```python
from build123d import *

# Parameters (mm, degrees)
CHAMFER1_SIZE  = 0.5
CHAMFER2_SIZE  = 1
CHAMFER2_SIZE2 = 0.3


with BuildPart() as part:
    # Sketch2 → Revolve1 (revolve)
    with BuildSketch(Plane.XY, mode=Mode.PRIVATE) as revolve1_sk:
        Polygon((4.5, 0), (4.5, 6), (4.9, 6), (4.9, 3), (6.25, 3), (6.25, 0), align=None)
    revolve(revolve1_sk.sketch.rotate(Axis((0, 0, 0), (0, 1, 0)), 90), axis=Axis((0, 0, 0), (0, 1, 0)))

    # Sketch3 → Cut-Revolve1 (revolve, cut)
    with BuildSketch(Plane.XY, mode=Mode.PRIVATE) as cut_revolve1_sk:
        Polygon((4.5, 3), (4.5, 0), (4.8, 0), align=None)
    revolve(cut_revolve1_sk.sketch.rotate(Axis((0, 0, 0), (0, 1, 0)), 90), axis=Axis((0, 0, 0), (0, 1, 0)), mode=Mode.SUBTRACT)

    # Chamfer1
    chamfer1_edges = [part.edges().sort_by_distance(p)[0] for p in [
        (0, 0, 6.25),
    ]]
    chamfer(chamfer1_edges, length=CHAMFER1_SIZE)

    # Chamfer2
    chamfer2_edges = [part.edges().sort_by_distance(p)[0] for p in [
        (0, 6, 4.5),
    ]]
    chamfer2_side = [part.faces().sort_by_distance(p)[0] for p in [
        (0, 4.5, 4.5),
    ]]
    chamfer(chamfer2_edges, length=CHAMFER2_SIZE, length2=CHAMFER2_SIZE2, reference=chamfer2_side[0])


solid = part.part
```
Design review of the part built by this model. Coordinates are the model's own, in mm. Coordinates: 2 decimals unless noted, no trailing zeros. Write each loop counter-clockwise with the first axis right and the second up, starting at its lowest first coordinate (ties: lowest second). Pieces come first, ordered by that corner, then holes.
1) Add section D-D (y = 2.7). Write out the cut boundary in (x, z), plus the area to 4 significant figures.
2) Add section B-B (x = 0). Write out the cut boundary in (y, z), plus the area to 4 significant figures.
3) Add section A-A (z = 0). Write out the cut boundary in (x, y), plus the area to 4 significant figures.
4) To check wall thickness, follow L1, parallel to X at y = 3.8, z = 0; L2, parallel to Y at x = 2.5, z = -5; L3, parallel to Z at x = 3, y = 4.5. State the ranges of each line that lie inside material, in increasing order.
5) Mouldability with a two-part tool opening along Z and no side actions: class faces 1 (the conical face through (4.5, 1.9, 1)), 2 (the cylindrical face through (-3.312, 4.479, 3.612)), 3 (the flat face through (2, 3, -5)) as +Z half, -Z half, draft (parallel to the pull), parting line (faces both ways), or undercut.
6) Add section C-C (y = 3.5). Write out the cut boundary in (x, z), plus the area to 3 significant figures.
7) Insertion check: pin 1 (1.5 mm diameter, centred on x = 3.5, z = 4.5, fed in from +Y); pin 2 (1 mm diameter, centred on y = 2, z = 4, fed in from -X); pin 3 (1.5 mm diameter, centred on y = 2, z = -2.5, fed in from +X). Each pin has a flat end and moves straight along its axis. Give the tip position at first contact, or say it passes through.
Check result:
1. outline: circle Ø12.5 at (0, 0); hole circle Ø9.06 at (0, 0)
1. area: 58.25 mm2
2. outline: (0, -5.75) - (0.5, -6.25) - (3, -6.25) - (3, -4.9) - (6, -4.9) - (6, -4.8) - (5, -4.5) - (3, -4.5) - (0, -4.8) - close; (0, 4.8) - (3, 4.5) - (5, 4.5) - (6, 4.8) - (6, 4.9) - (3, 4.9) - (3, 6.25) - (0.5, 6.25) - (0, 5.75) - close
2. area: 11.45 mm2
3. outline: (-6.25, 0.5) - (-5.75, 0) - (-4.8, 0) - (-4.5, 3) - (-4.5, 5) - (-4.8, 6) - (-4.9, 6) - (-4.9, 3) - (-6.25, 3) - close; (4.5, 3) - (4.8, 0) - (5.75, 0) - (6.25, 0.5) - (6.25, 3) - (4.9, 3) - (4.9, 6) - (4.8, 6) - (4.5, 5) - close
3. area: 11.45 mm2
4. L1: x = -4.9 to -4.5, 4.5 to 4.9
4. L2: y = 0 to 3
4. L3: z = -3.87 to -3.35, 3.35 to 3.87
5. face 1: undercut
5. face 2: parting line
5. face 3: draft
6. outline: circle Ø9.8 at (0, 0); hole circle Ø9 at (0, 0)
6. area: 11.8 mm2
7. pin 1: stops at y = 3
7. pin 2: stops at x = -5.18
7. pin 3: stops at x = 6
